Can you work these out from the model? Positions are in its coordinate system, mm. Coordinates: 2 decimals unless noted, no trailing zeros. Loops run counter-clockwise (first coordinate to the right, second up) from the corner with the lowest first, then second, coordinate; pieces in that order, holes last. Notation, with made-up numbers: (-6, -35.5) -> (34, -35.5) arc R38 ccw to (34, 2.5) -> close; hole circle Ø11 at (4, 88.25). An arc over 180 degrees is marked (long way). Use one line per item in the form item = value. Start each with the question number.
(1) Imagine slicing it at A-A (x = -17.5). List the corners of the cut face in (y, z) for me.
(2) Imagine slicing it at B-B (z = 0.7). List the corners of the cut face in (x, y) for me, plus the area to 3 significant figures.
(3) I'm going to push flat-ended pins straight in: pin 1 (6.5 mm diameter, centred on x = 17.5, y = -17.5, fed in from -Z); pin 2 (4.5 mm diameter, centred on x = 17.5, y = 17.5, fed in from +Z); pin 3 (3 mm diameter, centred on x = 5.5, y = -20.5, fed in from -Z); pin 4 (6 mm diameter, centred on x = -17.5, y = -17.5, fed in from -Z). Where does each tip first touch, or does it pass through?
(4) Thinking about a two-plate mould opening in Y: for faces 1 (the conical face through (-14.966, -16.702, 2.093)), 2 (the flat face through (27.5, 0, 2)), 3 (the flat face through (0, -27.5, 2)), which applies, released by +Y, released by -Y, zero draft, split by the parting line, or undercut?
(5) I need wall thicknesses on line 1 (Y direction, x = -17.5, z = 3.4); line 2 (X direction, y = 15.5, z = 0.8); line 3 (X direction, y = -21, z = 0.65). Which ranges of each line are inside material? Lowest first, please. Write a range as [from, to].
```python
from build123d import *

# Parameters (mm, degrees)
SKETCH1_W                  = 55
SKETCH1_H                  = 55
SKETCH1_W_2                = 35
SKETCH1_H_2                = 35
BOSS_EXTRUDE1_DEPTH        = 4
F_1_0_5_1_DIAMETER_HOLE1_D = 5.1
CHAMFER1_SIZE              = 2.2


with BuildPart() as part:
    # Sketch1 → Boss-Extrude1 (new body)
    # profile 1 of 2: a face of its own
    with BuildSketch(Plane.XY):
        Rectangle(SKETCH1_W, SKETCH1_H)
        Rectangle(SKETCH1_W_2, SKETCH1_H_2, mode=Mode.SUBTRACT)
    # profile 2 of 2: a face of its own
    with BuildSketch(Plane.XY):
        Rectangle(SKETCH1_W_2, SKETCH1_H_2)
    extrude(amount=BOSS_EXTRUDE1_DEPTH)

    # Ø1.0 (5.1) Diameter Hole1 (through all)
    with Locations(Plane(origin=(0, 0, 0), x_dir=(-1, 0, 0), z_dir=(0, 0, -1))):
        with Locations((-17.5, 17.5), (17.5, 17.5), (17.5, -17.5), (-17.5, -17.5)):
            Hole(F_1_0_5_1_DIAMETER_HOLE1_D / 2)

    # Chamfer1
    chamfer1_edges = [part.edges().sort_by_distance(p)[0] for p in [
        (14.95, -17.5, 0),
        (-20.05, -17.5, 0),
        (-20.05, 17.5, 0),
        (14.95, 17.5, 0),
    ]]
    chamfer(chamfer1_edges, length=CHAMFER1_SIZE)


solid = part.part
```
Worked out:
q1.outline = (-27.5, 0) -> (-22.25, 0) -> (-20.05, 2.2) -> (-20.05, 4) -> (-27.5, 4) -> close; (-14.95, 2.2) -> (-12.75, 0) -> (12.75, 0) -> (14.95, 2.2) -> (14.95, 4) -> (-14.95, 4) -> close; (20.05, 2.2) -> (22.25, 0) -> (27.5, 0) -> (27.5, 4) -> (20.05, 4) -> close
q2.outline = (-27.5, -27.5) -> (27.5, -27.5) -> (27.5, 27.5) -> (-27.5, 27.5) -> close; hole circle Ø8.1 at (-17.5, -17.5); hole circle Ø8.1 at (-17.5, 17.5); hole circle Ø8.1 at (17.5, -17.5); hole circle Ø8.1 at (17.5, 17.5)
q2.area = 2,820 mm2
q3.pin_1 = 1.5
q3.pin_2 = through
q3.pin_3 = 0
q3.pin_4 = 1.75
q4.face_1 = undercut
q4.face_2 = zero draft
q4.face_3 = released by -Y
q5.line_1 = [-27.5, -20.05], [-14.95, 14.95], [20.05, 27.5]
q5.line_2 = [-27.5, -20.91], [-14.09, 14.09], [20.91, 27.5]
q5.line_3 = [-27.5, -19.64], [-15.36, 15.36], [19.64, 27.5]
